Verification items for the finished model (mm, model axes). A direction names the side the tool comes from. Round coordinates to 2 decimals unless told otherwise and drop trailing zeros. Write each loop counter-clockwise with the first axis right and the second up, starting at its lowest first coordinate (ties: lowest second). Pieces come first, ordered by that corner, then holes.
from build123d import *


with BuildPart() as part:
    # Sketch2 → Revolve1 (revolve)
    with BuildSketch(Plane.XY):
        Polygon((25, 0), (29, 0), (29, 5), (28, 5), (24.75, 6.5), (24.25, 6.5), (25, 5), align=None)
    revolve(axis=Axis((0, -1000, 0), (0, 1, 0)))


solid = part.part
Q1. Release check for a two-part mould opening along Z. For faces 1 (the cylindrical face through (23.846, 2.465, -7.509)), 2 (the conical face through (-5.4, 6.427, 24.316)), 3 (the flat face through (16.4, 6.5, 18.2)) record: released by +Z, released by -Z, zero draft, split by the parting line, or undercut.
Recorded:
face 1: undercut
face 2: split by the parting line
face 3: zero draft
Q2. Depth check by flat-ended pin: P1, Ø1.5, axis at x = 7, y = 2.5, coming from the +Z side. Enter the tip coordinate at first touch or a pass-through.
Recorded:
P1: stops at z = 28.32
Q3. Material ranges on line 1 along X through (y, z) = (1.1, 0); line 2 along X through (y, z) = (2.5, 14), recorded low to high.
Recorded:
line 1: x = -29 to -25, 25 to 29
line 2: x = -25.4 to -20.71, 20.71 to 25.4
Q4. Sectioned sample at C-C (y = 4.25). Enter the section's corners in (x, z), plus the area to 3 significant figures.
Recorded:
outline: circle Ø58 at (0, 0); hole circle Ø50 at (0, 0)
area: 679 mm2
Q5. Sectioned sample at B-B (z = 0). Enter the section's corners in (x, y).
Recorded:
outline: (-29, 0) - (-25, 0) - (-25, 5) - (-24.25, 6.5) - (-24.75, 6.5) - (-28, 5) - (-29, 5) - close; (24.25, 6.5) - (25, 5) - (25, 0) - (29, 0) - (29, 5) - (28, 5) - (24.75, 6.5) - close
Q6. Tool access check on faces 4 (the cylindrical face through (13.38, 2.54, 25.73)), 5 (the flat face through (-15, 5, -24)). Record the directions out of +Z, -Z, +X, -X, +Y, -Y that give a thin tool (end or side, any length) a straight path to the whole face; none if there is none.
Recorded:
face 4: +Y, -Y
face 5: +Y
Q7. Sectioned sample at A-A (x = 0). Enter the section's corners in (y, z).
Recorded:
outline: (0, -29) - (5, -29) - (5, -28) - (6.5, -24.75) - (6.5, -24.25) - (5, -25) - (0, -25) - close; (0, 25) - (5, 25) - (6.5, 24.25) - (6.5, 24.75) - (5, 28) - (5, 29) - (0, 29) - close
